from build123d import *

# Parameters (mm, degrees)
SKETCH2_OUTSIDE_W = 81.556
SKETCH2_OUTSIDE_H = 81.556
CUT_EXTRUDE_DEPTH = 47.45561719
SKETCH4_W         = 5.7
SKETCH4_H         = 3.5
EXTRUDE1_DEPTH    = 1.5


with BuildPart() as part:
    # Sketch1 → Base-Extrude (revolve)
    with BuildSketch(Plane.YZ, mode=Mode.PRIVATE) as base_extrude_sk:
        Polygon((0, -4.247960103), (-24.5, -4.247960103), (-31, -1.371705006), (-30.393019459, 0), (-24.5, -2.747960103), (0, -2.747960103), align=None)
    revolve(base_extrude_sk.sketch.rotate(Axis((0, 0, 5.823648763), (0, 0, -1)), 270), axis=Axis((0, 0, 5.823648763), (0, 0, -1)))

    # Sketch2 outside → Cut-Extrude (cut, through all)
    # profile 1 of 2: a face of its own
    with BuildSketch(Plane(origin=(-2.40435344, 1.003568156, -4.247960103), x_dir=(-1, 0, 0), z_dir=(0, 0, -1))):
        with Locations((-2.404, -1.004)):
            Rectangle(SKETCH2_OUTSIDE_W, SKETCH2_OUTSIDE_H)
        with BuildLine():
            Line((-26.738023529, -3.853568156), (-33.273067375, -3.853568156))
            ThreePointArc((-33.273067375, -3.853568156), (-33.40435344, -1.003568156), (-33.273067375, 1.846431844))
            Line((-33.273067375, 1.846431844), (-26.738023529, 1.846431844))
            ThreePointArc((-26.738023529, 1.846431844), (-26.069536184, 5.337498449), (-24.902929904, 8.695094487))
            Line((-24.902929904, 8.695094487), (-30.562443889, 11.96261641))
            ThreePointArc((-30.562443889, 11.96261641), (-29.251140957, 14.496431844), (-27.712443889, 16.898961212))
            Line((-27.712443889, 16.898961212), (-22.052929904, 13.631439289))
            ThreePointArc((-22.052929904, 13.631439289), (-19.728469579, 16.320547983), (-17.039360885, 18.645008308))
            Line((-17.039360885, 18.645008308), (-20.306882808, 24.304522293))
            ThreePointArc((-20.306882808, 24.304522293), (-17.90435344, 25.843219361), (-15.370538006, 27.154522293))
            Line((-15.370538006, 27.154522293), (-12.103016083, 21.495008308))
            ThreePointArc((-12.103016083, 21.495008308), (12.510301571, 18.433588681), (21.837801226, -4.548696808))
            Line((21.837801226, -4.548696808), (28.150168853, -6.240090616))
            ThreePointArc((28.150168853, -6.240090616), (27.539347175, -9.026958555), (26.674900296, -11.745867825))
            Line((26.674900296, -11.745867825), (20.362532669, -10.054474018))
            ThreePointArc((20.362532669, -10.054474018), (18.813268953, -13.253568156), (16.817404018, -16.194816961))
            Line((16.817404018, -16.194816961), (21.438377837, -20.81579078))
            ThreePointArc((21.438377837, -20.81579078), (19.515956777, -22.923878373), (17.407869184, -24.846299433))
            Line((17.407869184, -24.846299433), (12.786895365, -20.225325614))
            ThreePointArc((12.786895365, -20.225325614), (9.84564656, -22.221190549), (6.646552422, -23.770454265))
            Line((6.646552422, -23.770454265), (8.33794623, -30.082821892))
            ThreePointArc((8.33794623, -30.082821892), (5.619036959, -30.947268771), (2.83216902, -31.558090449))
            Line((2.83216902, -31.558090449), (1.140775212, -25.245722822))
            ThreePointArc((1.140775212, -25.245722822), (-17.31900845, -20.440724994), (-26.738023529, -3.853568156))
        make_face(mode=Mode.SUBTRACT)
    # profile 2 of 2: a face of its own
    with BuildSketch(Plane(origin=(-2.40435344, 1.003568156, -4.247960103), x_dir=(-1, 0, 0), z_dir=(0, 0, -1))):
        with BuildLine():
            Line((-22.452794776, 1.846431844), (-19.15435344, 1.846431844))
            Line((-19.15435344, 1.846431844), (-19.15435344, -3.853568156))
            Line((-19.15435344, -3.853568156), (-22.452794776, -3.853568156))
            ThreePointArc((-22.452794776, -3.853568156), (17.84564656, -1.003568156), (-22.452794776, 1.846431844))
        make_face()
    extrude(amount=-CUT_EXTRUDE_DEPTH, mode=Mode.SUBTRACT)

    # Sketch4 → Extrude1 (add)
    with BuildSketch(Plane(origin=(16.75, -0.667304961, -0.255028377), x_dir=(0, 1, 0), z_dir=(-1, 0, 0))):
        with Locations((0.667304961, 0.742931726)):
            Rectangle(SKETCH4_W, SKETCH4_H)
    extrude(amount=-EXTRUDE1_DEPTH)


solid = part.part
Can you work these out from the model? Positions are in its coordinate system, mm. A direction names the side the tool comes from. Round coordinates to 2 decimals unless told otherwise and drop trailing zeros. Order: outer loops, then holes, each group sorted by start corner. A loop starts at its lowest first (then second) coordinate and runs counter-clockwise, first axis right, second up. Notation, with made-up numbers: M 37.25,16 L 54.25,16 A15 ccw 54.25,24 Z; hole C 54,-39.5 d3. An arc over 180 degrees is marked long. Use a Markdown table: item, result.
1) On a 3-axis mill with a long thin cutter (end or side, diameter ignored), from which of +Z, -Z, +X, -X, +Y, -Y can I reach the whole of each face in a straight line? I mean faces 1 (the face through (27.41, 0.04, -1.39)), 2 (the face through (16.246, 22.439, -2.154)), 3 (the face through (-19.35, -19.41, -1.39)), 4 (the face through (-21.5, -17.47, -2.15)). Say none if no direction works.
Geometry says:
| item | result |
|---|---|
| face 1 | +Z |
| face 2 | +Z, -Z, +X |
| face 3 | +Z, +X, +Y |
| face 4 | +Z, -Z, -X |
2) Imagine slicing it at D-D (y = 7). List the corners of the cut face in (x, z) for me, then the cut area to 3 significant figures.
Geometry says:
| item | result |
|---|---|
| outline | M -23.48,-4.25 L -19,-4.25 L -19,-2.75 L -23.48,-2.75 Z; M 19,-4.25 L 23.48,-4.25 L 23.48,-2.75 L 19,-2.75 Z |
| area | 13.4 mm² |
3) Imagine slicing it at A-A (x = 0). List the corners of the cut face in (y, z) for me.
Geometry says:
| item | result |
|---|---|
| outline | M -24.5,-4.25 L -20.25,-4.25 L -20.25,-2.75 L -24.5,-2.75 Z; M 20.25,-4.25 L 24.5,-4.25 L 24.5,-2.75 L 20.25,-2.75 Z |
4) If we mould it in two halves opening along X, with no side actions, what happens to faces 5 (the face through (-7.9, -29.66, -0.68)), 6 (the face through (16.75, 0, -2)), 7 (the face through (18, -2, -4.248))? For each: +X half, -X half, draft (parallel to the pull), parting line (faces both ways), or undercut.
Geometry says:
| item | result |
|---|---|
| face 5 | -X half |
| face 6 | undercut |
| face 7 | draft |
5) If I drill on line 1 along Y through (x, z) = (0, -3.45); line 2 along Z through (x, y) = (17.5, 16); line 3 along X through (y, z) = (0, -3.7), over which ranges is the centre line in solid material (lowest first)?
Geometry says:
| item | result |
|---|---|
| line 1 | y = -24.5 to -20.25, 20.25 to 24.5 |
| line 2 | z = -4.25 to -2.75 |
| line 3 | x = -24.5 to -20.25, 16.75 to 25.74 |
6) Imagine slicing it at B-B (y = 0). List the corners of the cut face in (x, z) for me.
Geometry says:
| item | result |
|---|---|
| outline | M -24.5,-4.25 L -20.25,-4.25 L -20.25,-2.75 L -24.5,-2.75 Z; M 16.75,-4.25 L 24.5,-4.25 L 31,-1.37 L 30.39,0 L 24.5,-2.75 L 18.25,-2.75 L 18.25,0.75 L 16.75,0.75 Z |
7) I'm going to push flat-ended pins straight in: P1, Ø2, axis at y = -8.5, z = -2.5, coming from the +X side; P2, Ø1, axis at x = 19, z = -1.5, coming from the -Y side; P3, Ø3, axis at y = 0.5, z = -0.5, coming from the +X side; P4, Ø2.5, axis at y = 0.5, z = -1, coming from the -X side. Where does each tip first touch, or does it pass through?
Geometry says:
| item | result |
|---|---|
| P1 | stops at x = 23.31 |
| P2 | passes through |
| P3 | stops at x = 31 |
| P4 | stops at x = 16.75 |
